Read the model definition and answer for the solid it produces. Units are mm, in the model's axes. A direction names the side the tool comes from. Give positions to 0.01 mm unless a question says otherwise; leave off trailing zeros. Order: outer loops, then holes, each group sorted by start corner. A loop starts at its lowest first (then second) coordinate and runs counter-clockwise, first axis right, second up. Notation, with made-up numbers: (-33.75, 33) - (-13.75, 33) arc R25 cw to (-13.75, 63) - close; hole circle Ø8 at (59.5, -3). An arc over 180 degrees is marked (long way). Return JSON: item names as keys, results as strings.
```python
from build123d import *

# Parameters (mm, degrees)
SKETCH1_W                                            = 32
SKETCH1_H                                            = 32
BOSS_EXTRUDE1_DEPTH                                  = 7.5
SKETCH2_R                                            = 10
CUT_EXTRUDE1_DEPTH                                   = 28.147743921
SKETCH3_R                                            = 12
CUT_EXTRUDE2_DEPTH                                   = 5
CUT_EXTRUDE3_START                                   = -7
SKETCH4_R                                            = 12
CUT_EXTRUDE3_DEPTH                                   = 7
CHAMFER1_SIZE                                        = 2
HOLE_SIZE_PER_SOCKET_HEAD_CAP_SCREW_TYPE_D           = 3.5
HOLE_SIZE_PER_SOCKET_HEAD_CAP_SCREW_TYPE_CBORE_D     = 6
HOLE_SIZE_PER_SOCKET_HEAD_CAP_SCREW_TYPE_CBORE_DEPTH = 4


with BuildPart() as part:
    # Sketch1 → Boss-Extrude1 (new, symmetric)
    with BuildSketch(Plane.XY):
        Rectangle(SKETCH1_W, SKETCH1_H)
    extrude(amount=BOSS_EXTRUDE1_DEPTH, both=True)

    # Sketch2 → Cut-Extrude1 (cut, through all)
    with BuildSketch(Plane.XY.offset(7.5)):
        Circle(SKETCH2_R)
    extrude(amount=-CUT_EXTRUDE1_DEPTH, mode=Mode.SUBTRACT)

    # Sketch3 → Cut-Extrude2 (cut)
    with BuildSketch(Plane.XY.offset(7.5)):
        Circle(SKETCH3_R)
    extrude(amount=-CUT_EXTRUDE2_DEPTH, mode=Mode.SUBTRACT)

    # Sketch4 → Cut-Extrude3 (cut)
    with BuildSketch(Plane(origin=(0, 0, -7.5), x_dir=(-1, 0, 0), z_dir=(0, 0, -1)).offset(CUT_EXTRUDE3_START)):
        with Locations(Location((0, 0, 0), (0, 0, 180))):
            Circle(SKETCH4_R)
    extrude(amount=CUT_EXTRUDE3_DEPTH, mode=Mode.SUBTRACT)

    # Chamfer1
    chamfer1_edges = [part.edges().sort_by_distance(p)[0] for p in [
        (16, -16, 0),
        (-16, -16, 0),
        (-16, 16, 0),
        (16, 16, 0),
    ]]
    chamfer(chamfer1_edges, length=CHAMFER1_SIZE)

    # Hole size per socket head cap screw type1 (through all)
    with Locations(Plane.XY.offset(7.5)):
        with Locations((-12, 12), (12, 12), (12, -12), (-12, -12)):
            CounterBoreHole(HOLE_SIZE_PER_SOCKET_HEAD_CAP_SCREW_TYPE_D / 2, HOLE_SIZE_PER_SOCKET_HEAD_CAP_SCREW_TYPE_CBORE_D / 2, HOLE_SIZE_PER_SOCKET_HEAD_CAP_SCREW_TYPE_CBORE_DEPTH)


solid = part.part
```
Q1. A cutting plane is placed at C-C (x = -4). Write down the section's boundary in (y, z), and give its area (3 significant figures).
Values:
{"outline": "(-16, -7.5) - (-11.31, -7.5) - (-11.31, -0.5) - (-9.17, -0.5) - (-9.17, 2.5) - (-11.31, 2.5) - (-11.31, 7.5) - (-16, 7.5) - close; (9.17, -0.5) - (11.31, -0.5) - (11.31, -7.5) - (16, -7.5) - (16, 7.5) - (11.31, 7.5) - (11.31, 2.5) - (9.17, 2.5) - close", "area": "153 mm²"}
Q2. Determine the mould class of faces 4 (the flat face through (16, 0, 0)), 5 (the cylindrical face through (-13.669, 12.526, -2.077)), 6 (the flat face through (-10, -12, 3.5)), 7 (the flat face through (0, -16, 0)) for opening direction X: released by +X, released by -X, zero draft, split by the parting line, or undercut.
Values:
{"face 4": "released by +X", "face 5": "undercut", "face 6": "undercut", "face 7": "zero draft"}
Q3. For faces 1 (the flat face through (0, 16, 0)), 2 (the cylindrical face through (9.6, 10.2, 5.5)), 3 (the cylindrical face through (11.446, -3.604, -3.951)), determine the directions among +Z, -Z, +X, -X, +Y, -Y from which every point of the face is accessible in a straight line to the end or side of a thin tool.
Values:
{"face 1": "+Z, -Z, +X, -X, +Y", "face 2": "+Z", "face 3": "-Z"}
Q4. Consider L1, parallel to Y at x = 12, z = 0.5; L2, parallel to X at y = 14, z = 7; L3, parallel to Z at x = 10.5, y = -1. Determine where each line is inside the solid, lowest interval first.
Values:
{"L1": "y = -16 to -13.75, -10.25 to 10.25, 13.75 to 16", "L2": "x = -16 to -14.24, -9.76 to 9.76, 14.24 to 16", "L3": "z = -0.5 to 2.5"}
Q5. Given pin 1 (5.5 mm diameter, centred on x = 12, y = -12, fed in from +Z); pin 2 (12 mm diameter, centred on x = -2.5, y = -4.5, fed in from -Z), each flat-ended and moving along its own axis, determine where each tip first touches the part or whether it passes through.
Values:
{"pin 1": "stops at z = 3.5", "pin 2": "stops at z = -0.5"}
Q6. A cutting plane is placed at D-D (y = -9.5). Write down the section's boundary in (x, z), and give its area (3 significant figures).
Values:
{"outline": "(-16, -7.5) - (-7.33, -7.5) - (-7.33, -0.5) - (-3.12, -0.5) - (-3.12, 2.5) - (-7.33, 2.5) - (-7.33, 7.5) - (-10.34, 7.5) - (-10.34, 3.5) - (-13.66, 3.5) - (-13.66, 7.5) - (-16, 7.5) - close; (3.12, -0.5) - (7.33, -0.5) - (7.33, -7.5) - (16, -7.5) - (16, 7.5) - (13.66, 7.5) - (13.66, 3.5) - (10.34, 3.5) - (10.34, 7.5) - (7.33, 7.5) - (7.33, 2.5) - (3.12, 2.5) - close", "area": "259 mm²"}
Q7. A cutting plane is placed at B-B (z = -5). Write down the section's boundary in (x, y).
Values:
{"outline": "(-16, -14) - (-14, -16) - (14, -16) - (16, -14) - (16, 14) - (14, 16) - (-14, 16) - (-16, 14) - close; hole circle Ø3.5 at (-12, -12); hole circle Ø3.5 at (-12, 12); hole circle Ø24 at (0, 0); hole circle Ø3.5 at (12, -12); hole circle Ø3.5 at (12, 12)"}
Q8. A cutting plane is placed at A-A (y = 0). Write down the section's boundary in (x, z), and give its area (3 significant figures).
Values:
{"outline": "(-16, -7.5) - (-12, -7.5) - (-12, -0.5) - (-10, -0.5) - (-10, 2.5) - (-12, 2.5) - (-12, 7.5) - (-16, 7.5) - close; (10, -0.5) - (12, -0.5) - (12, -7.5) - (16, -7.5) - (16, 7.5) - (12, 7.5) - (12, 2.5) - (10, 2.5) - close", "area": "132 mm²"}
